Print and shaded views of the part. All mm, measured from the part's lowest x, y and z. A direction names the side the tool comes from. Round coordinates to 2 decimals unless told otherwise and drop trailing zeros. Write each loop counter-clockwise with the first axis right and the second up, starting at its lowest first coordinate (ties: lowest second). Pieces come first, ordered by that corner, then holes. Notation, with made-up numbers: M -4.5,58 L 6.5,58 A21 ccw 6.5,93 Z; hole C 50,86.5 d5. An arc over 180 degrees is marked long. Write item = value, one per line. Start each with the question number.
Q1. Band-saw the part on D-D on y = 2.5. Write the cut outline in (x, z), plus the area to 3 significant figures.
Q2. Probe L1, parallel to Z at x = 15.5, y = 23.5; L2, parallel to X at y = 13.25, z = 38 (1 decimal); L3, parallel to Y at x = 10, z = 28.5. List the from-to ranges inside material, lowest first.
Q3. Band-saw the part on A-A on y = 8.25. Write the cut outline in (x, z).
Q4. Band-saw the part on B-B on z = 34.5. Write the cut outline in (x, y) (1 decimal).
Q5. Drop flat-ended pins along their axis: P1, Ø3, axis at y = 16.5, z = 45, coming from the +X side (1 decimal); P2, Ø1.5, axis at y = 18.5, z = 13, coming from the -X side; P3, Ø6, axis at x = 3.5, y = 3.5, coming from the +Z side. Give the stop position or say it passes through.
Q6. Band-saw the part on C-C on x = 16. Write the cut outline in (y, z) (1 decimal), plus the area to 3 significant figures.
Q7. Tool access for the marked faces 1, 2 and 3: list every direction of +Z, -Z, +X, -X, +Y, -Y with a clear straight run to the whole face (end or side of a thin tool).
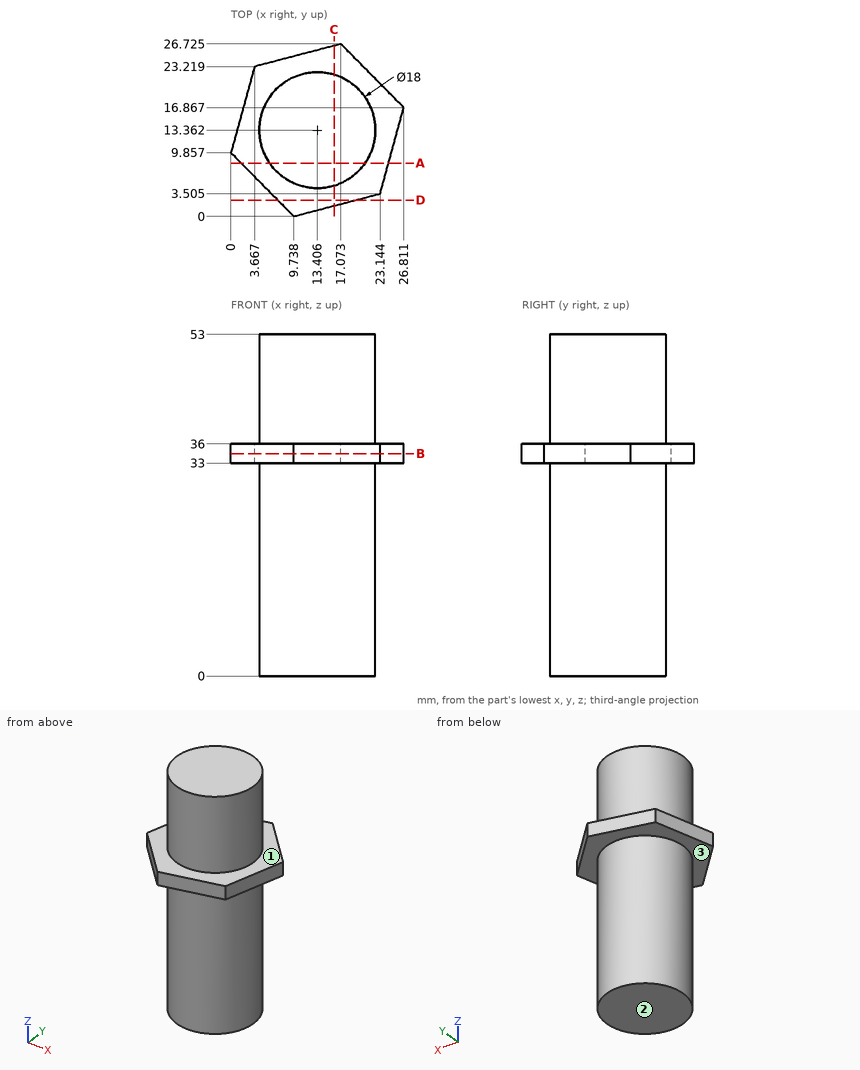
Conclusion:
q1.outline = M 7.27,33 L 19.3,33 L 19.3,36 L 7.27,36 Z
q1.area = 36.1 mm^2
q2.L1 = 33 to 36
q2.L2 = 4.4 to 22.4
q2.L3 = 5.03 to 21.69
q3.outline = M 1.59,33 L 6,33 L 6,0 L 20.81,0 L 20.81,33 L 24.45,33 L 24.45,36 L 20.81,36 L 20.81,53 L 6,53 L 6,36 L 1.59,36 Z
q4.outline = M 0,9.9 L 9.7,0 L 23.1,3.5 L 26.8,16.9 L 17.1,26.7 L 3.7,23.2 Z
q5.P1 = 22.3
q5.P2 = 5.55
q5.P3 = 36
q6.outline = M 1.6,33 L 4.7,33 L 4.7,0 L 22,0 L 22,33 L 26.4,33 L 26.4,36 L 22,36 L 22,53 L 4.7,53 L 4.7,36 L 1.6,36 Z
q6.area = 936 mm^2
q7.face_1 = +Z
q7.face_2 = -Z, +X, -X, +Y, -Y
q7.face_3 = -Z
